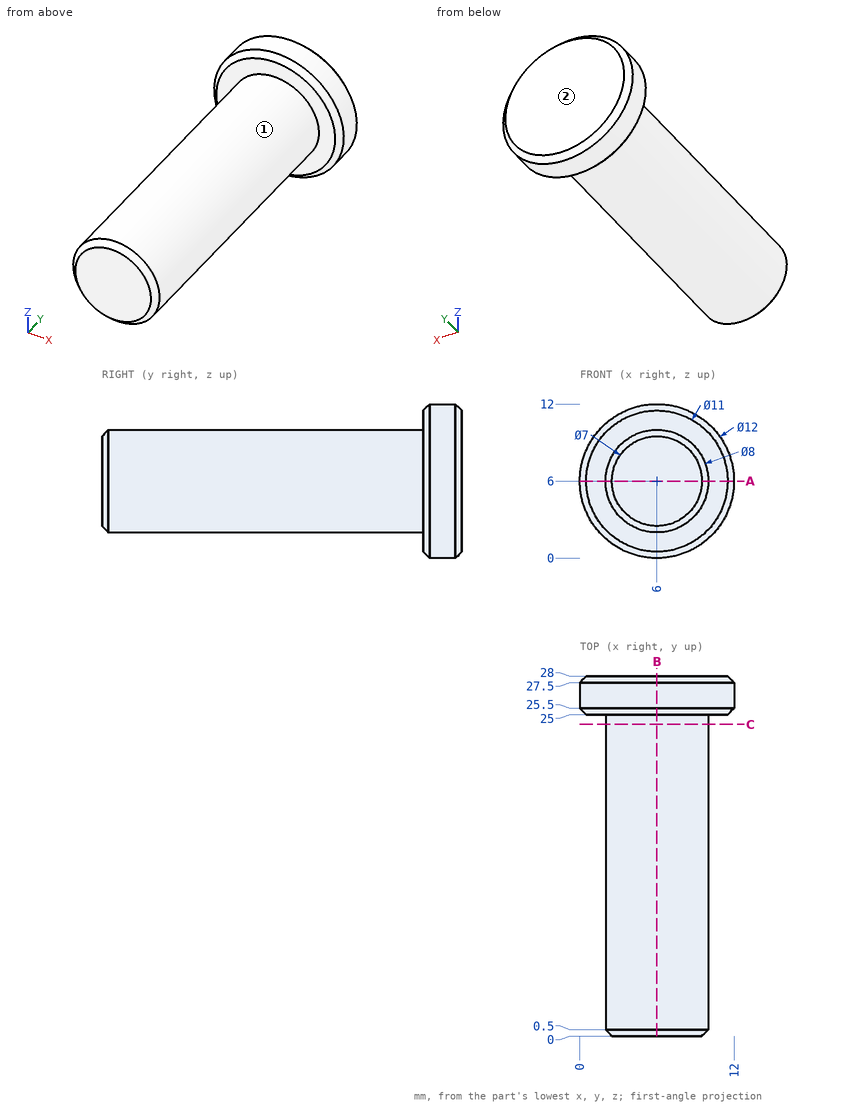
Could you check a few things on this drawing? It's one solid part, dimensions in mm from its lowest x, y, z. A direction names the side the tool comes from. Coordinates: 2 decimals unless noted, no trailing zeros. Order: outer loops, then holes, each group sorted by start corner. A loop starts at its lowest first (then second) coordinate and runs counter-clockwise, first axis right, second up. Notation, with made-up numbers: (75.25, 88.5) -> (123.25, 88.5) arc R11 cw to (123.25, 98.5) -> close; hole circle Ø5 at (-11, 50). An arc over 180 degrees is marked (long way). Answer in a Markdown table with one row per item.
(1) On a 3-axis mill with a long thin cutter (end or side, diameter ignored), from which of +Z, -Z, +X, -X, +Y, -Y can I reach the whole of each face in a straight line? I mean the marked faces 1 and 2. Say none if no direction works.
Answer key:
| item | result |
|---|---|
| face 1 | -Y |
| face 2 | +Z, -Z, +X, -X, +Y |
(2) Please list where these lines run through material, in increasing order: probe 1 along Y at (x, z) = (9.25, 3.25); probe 2 along X at (y, z) = (15, 9); probe 3 along X at (y, z) = (19.25, 4).
Answer key:
| item | result |
|---|---|
| probe 1 | 25 to 28 |
| probe 2 | 3.35 to 8.65 |
| probe 3 | 2.54 to 9.46 |
(3) I want a section at C-C on y = 24.25. List the corners of the cut face in (x, z) for me, then the cut area to 3 significant figures.
Answer key:
| item | result |
|---|---|
| outline | circle Ø8 at (6, 6) |
| area | 50.3 mm^2 |
(4) I want a section at B-B on x = 6. List the corners of the cut face in (y, z) for me.
Answer key:
| item | result |
|---|---|
| outline | (0, 2.5) -> (0.5, 2) -> (25, 2) -> (25, 0.5) -> (25.5, 0) -> (27.5, 0) -> (28, 0.5) -> (28, 11.5) -> (27.5, 12) -> (25.5, 12) -> (25, 11.5) -> (25, 10) -> (0.5, 10) -> (0, 9.5) -> close |
(5) I want a section at A-A on z = 6. List the corners of the cut face in (x, y) for me.
Answer key:
| item | result |
|---|---|
| outline | (0, 25.5) -> (0.5, 25) -> (2, 25) -> (2, 0.5) -> (2.5, 0) -> (9.5, 0) -> (10, 0.5) -> (10, 25) -> (11.5, 25) -> (12, 25.5) -> (12, 27.5) -> (11.5, 28) -> (0.5, 28) -> (0, 27.5) -> close |
(6) Will these pins go through, and if not, where does the flat tip stop? pin 1 Ø4 at (y, z) = (9, 4.5) entering from +X; pin 2 Ø5 at (y, z) = (17, 9.5) entering from -X; pin 3 Ø2 at (y, z) = (7.5, 8.5) entering from -X.
Answer key:
| item | result |
|---|---|
| pin 1 | x = 10 |
| pin 2 | x = 2.13 |
| pin 3 | x = 2.29 |
